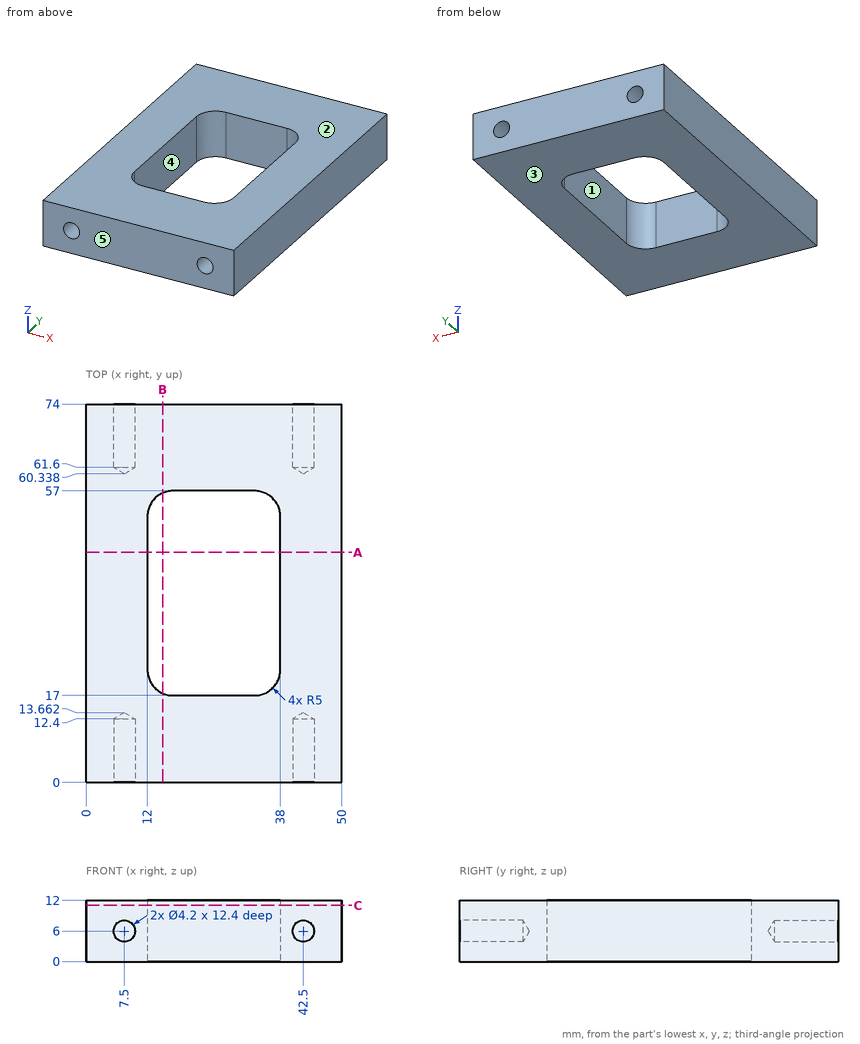
Study the drawing (mm; zero at the part's minimum x, y, z) and answer. A direction names the side the tool comes from. Round coordinates to 2 decimals unless told otherwise and drop trailing zeros. Write each loop counter-clockwise with the first axis right and the second up, starting at its lowest first coordinate (ties: lowest second). Pieces come first, ordered by that corner, then holes. Notation, with made-up numbers: (57, 48) - (112, 48) arc R30 cw to (112, 71) - close; hole circle Ø7 at (40.25, 22). An arc over 180 degrees is marked (long way). Return JSON: item names as keys, results as strings. Group by question number.
Q1. The part is cut by section C-C on z = 11. Write down the section's boundary in (x, y), then the cut area to 3 significant figures.
Q2. The mould has two halves that part along Y. Classify the marked faces 3, 4 and 5: released by +Y, released by -Y, zero draft, split by the parting line, or undercut.
Q3. For the marked faces 1 and 2, determine the directions among +Z, -Z, +X, -X, +Y, -Y from which every point of the face is accessible in a straight line to the end or side of a thin tool.
Q4. Each of these flat-tipped pins is pushed along its axis until it touches: pin 1 Ø3.5 at (x, z) = (7.5, 6) entering from -Y; pin 2 Ø2.5 at (x, z) = (42.5, 6) entering from -Y. Where does it stop, or does it pass through?
Q5. The part is cut by section B-B on x = 15. Write down the section's boundary in (y, z), then the cut area to 3 significant figures.
Q6. Find the intervals of material crossed by L1, parallel to X at y = 4.5, z = 6; L2, parallel to Y at x = 23.5, z = 7; L3, parallel to Z at x = 7.5, y = 4, in increasing order.
Q7. The part is cut by section A-A on y = 45. Write down the section's boundary in (x, z), then the cut area to 3 significant figures.
Solved:
{
 "1": {"outline": "(0, 0) - (50, 0) - (50, 74) - (0, 74) - close; hole (12, 22) arc R5 ccw to (17, 17) - (33, 17) arc R5 ccw to (38, 22) - (38, 52) arc R5 ccw to (33, 57) - (17, 57) arc R5 ccw to (12, 52) - close", "area": "2,680 mm²"},
 "2": {"face 3": "zero draft", "face 4": "undercut", "face 5": "released by -Y"},
 "3": {"face 1": "+Z, -Z", "face 2": "+Z, +X, -X, +Y, -Y"},
 "4": {"pin 1": "y = 12.61", "pin 2": "y = 12.91"},
 "5": {"outline": "(0, 0) - (17.42, 0) - (17.42, 12) - (0, 12) - close; (56.58, 0) - (74, 0) - (74, 12) - (56.58, 12) - close", "area": "418 mm²"},
 "6": {"L1": "0 to 5.4, 9.6 to 40.4, 44.6 to 50", "L2": "0 to 17, 57 to 74", "L3": "0 to 3.9, 8.1 to 12"},
 "7": {"outline": "(0, 0) - (12, 0) - (12, 12) - (0, 12) - close; (38, 0) - (50, 0) - (50, 12) - (38, 12) - close", "area": "288 mm²"}
}
